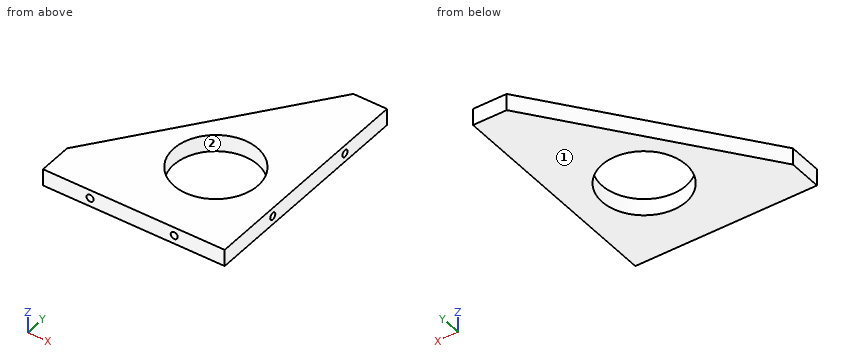
```python
from build123d import *

# Parameters (mm, degrees)
SKETCH_1_W             = 108
SKETCH_1_H             = 135
EXTRUDE_1_DEPTH        = 10
CUT_EXTRUDE_1_REACH    = 89.019
HOLE_WIZARD_M5_1_D     = 4.2
HOLE_WIZARD_M5_1_DEPTH = 12.4
HOLE_WIZARD_M5_1_TIP   = 1.2618073
HOLE_WIZARD_M5_2_D     = 4.2
HOLE_WIZARD_M5_2_DEPTH = 12.4
HOLE_WIZARD_M5_2_TIP   = 1.2618073
CUT_EXTRUDE_2_REACH    = 89.019
SKETCH_7_R             = 25


with BuildPart() as part:
    # 草图1 → 凸台-拉伸1 (new body)
    with BuildSketch(Plane.XY):
        Rectangle(SKETCH_1_W, SKETCH_1_H)
    extrude(amount=EXTRUDE_1_DEPTH)

    # 草图2 → 切除-拉伸1 (cut, up to next)
    with BuildSketch(Plane.XY.offset(10), mode=Mode.PRIVATE) as cut_extrude_1_sk1:
        Polygon((34, 67.5), (-54, 67.5), (-54, -47.5), align=None)
    cut_extrude_1_tool1 = extrude(cut_extrude_1_sk1.sketch, amount=-CUT_EXTRUDE_1_REACH, mode=Mode.PRIVATE) & part.part
    add(cut_extrude_1_tool1.solids().sort_by_distance((-24.666667, 29.166667, 10))[0], mode=Mode.SUBTRACT)

    # M5 螺纹孔1
    with Locations(Plane(origin=(0, -67.5, 0), x_dir=(-1, 0, 0), z_dir=(0, -1, 0))):
        with Locations((-24, -5), (26, -5)):
            Hole(HOLE_WIZARD_M5_1_D / 2, depth=HOLE_WIZARD_M5_1_DEPTH)
            with Locations((0, 0, -(HOLE_WIZARD_M5_1_DEPTH + HOLE_WIZARD_M5_1_TIP / 2))):  # 118° drill point
                Cone(0, HOLE_WIZARD_M5_1_D / 2, HOLE_WIZARD_M5_1_TIP, mode=Mode.SUBTRACT)

    # M5 螺纹孔2
    with Locations(Plane(origin=(54, 0, 0), x_dir=(0, 0, -1), z_dir=(1, 0, 0))):
        with Locations((-5, -27.5), (-5, 32.5)):
            Hole(HOLE_WIZARD_M5_2_D / 2, depth=HOLE_WIZARD_M5_2_DEPTH)
            with Locations((0, 0, -(HOLE_WIZARD_M5_2_DEPTH + HOLE_WIZARD_M5_2_TIP / 2))):  # 118° drill point
                Cone(0, HOLE_WIZARD_M5_2_D / 2, HOLE_WIZARD_M5_2_TIP, mode=Mode.SUBTRACT)

    # 草图7 → 切除-拉伸2 (cut, up to next)
    with BuildSketch(Plane(origin=(0, 0, 0), x_dir=(-1, 0, 0), z_dir=(0, 0, -1)), mode=Mode.PRIVATE) as cut_extrude_2_sk1:
        with Locations((-13.028146721, -17.5)):
            Circle(SKETCH_7_R)
    cut_extrude_2_tool1 = extrude(cut_extrude_2_sk1.sketch, amount=-CUT_EXTRUDE_2_REACH, mode=Mode.PRIVATE) & part.part
    add(cut_extrude_2_tool1.solids().sort_by_distance((13.028147, -17.5, 0))[0], mode=Mode.SUBTRACT)


solid = part.part
```
CAD build for the part. Positions are in the model's coordinates, mm. Face numbers are marked on the shaded views. Give positions to 0.01 mm unless a question says otherwise; leave off trailing zeros. Order: outer loops, then holes, each group sorted by start corner. A loop starts at its lowest first (then second) coordinate and runs counter-clockwise, first axis right, second up.
(1) Mould opens along X. For the marked faces 1 and 2 say: released by +X, released by -X, zero draft, split by the parting line, or undercut.
(2) Drill centre lines: L1, parallel to Y at x = 46.75, z = 5; L2, parallel to Z at x = 46.5, y = -27.5; L3, parallel to X at y = -55, z = 4.75. Where is each one in solid material? Low to high.
(3) Flat gauge pins, fed straight in: pin 1 (1 mm diameter, centred on x = -23, z = 6, fed in from +Y); pin 2 (3.5 mm diameter, centred on x = -26, z = 5, fed in from -Y); pin 3 (4 mm diameter, centred on x = 24, z = 5, fed in from +Y). Where does each tip first touch, or does it go through?
(4) Saw through at C-C, the plane y = 18.5. Give the cut face in (x, z).
(5) Saw through at A-A, the plane x = -1. Give the cut face in (y, z).
(6) Saw through at D-D, the plane x = -36. Give the cut face in (y, z).
(7) Saw through at B-B, the plane y = -17.5. Give the cut face in (x, z).
Results found:
1. face 1: zero draft
1. face 2: undercut
2. L1: y = -67.5 to -29.6, -25.4 to 30.4, 34.6 to 67.5
2. L2: z = 0 to 2.9, 7.1 to 10
2. L3: x = -54 to -27.92, -24.08 to 22.08, 25.92 to 54
3. pin 1: stops at y = -6.34
3. pin 2: stops at y = -54.89
3. pin 3: stops at y = 57.05
4. outline: (-3.5, 0) - (54, 0) - (54, 10) - (-3.5, 10) - close
5. outline: (-67.5, 0) - (-38.19, 0) - (-38.19, 10) - (-67.5, 10) - close; (3.19, 0) - (21.76, 0) - (21.76, 10) - (3.19, 10) - close
6. outline: (-67.5, 0) - (-23.98, 0) - (-23.98, 10) - (-67.5, 10) - close
7. outline: (-31.04, 0) - (-11.97, 0) - (-11.97, 10) - (-31.04, 10) - close; (38.03, 0) - (54, 0) - (54, 10) - (38.03, 10) - close
